Geometry: final body of the model. Coordinates: model frame, mm. A direction names the side the tool comes from. Give positions to 0.01 mm unless a question says otherwise; leave off trailing zeros. Write each loop counter-clockwise with the first axis right and the second up, starting at its lowest first coordinate (ties: lowest second). Pieces come first, ordered by that corner, then holes. Notation, with made-up numbers: (-34, 80) - (-20, 80) arc R7 ccw to (-20, 92) - close; hole circle Ø8 at (-14, 65). An arc over 180 degrees is marked (long way). One line per question, with ' | ' between items. Start each with the question number.
```python
from build123d import *

# Parameters (mm, degrees)
CHAMFER1_SIZE       = 5
SKETCH3_W           = 40
SKETCH3_H           = 200
BOSS_EXTRUDE1_DEPTH = 5
SKETCH4_W           = 500
SKETCH4_H           = 129
BOSS_EXTRUDE2_DEPTH = 10
CIRPATTERN2_COUNT   = 4


with BuildPart() as part:
    # Sketch2 → Revolve1 (revolve)
    with BuildSketch(Plane(origin=(0, 0, 0), x_dir=(1, 0, 0), z_dir=(0, 1, 0))):
        Polygon((-55.931623932, 0), (-55.931623932, 8), (-20.931623932, 8), (-20.931623932, 11), (-13.931623932, 11), (-13.931623932, 12.5), (26.068376068, 12.5), (26.068376068, 30), (568.068376068, 30), (568.068376068, 12.5), (594.068376068, 12.5), (594.068376068, 0), align=None)
    revolve(axis=Axis((0, 0, 0), (-1, 0, 0)))

    # Chamfer1
    chamfer1_edges = [part.edges().sort_by_distance(p)[0] for p in [
        (26.068376068, 0, 30),
        (568.068376068, 0, 30),
    ]]
    chamfer(chamfer1_edges, length=CHAMFER1_SIZE)

    # Sketch3 → Boss-Extrude1 (add, symmetric)
    with BuildSketch(Plane.XY):
        with Locations((139.068376068, 100)):
            Rectangle(SKETCH3_W, SKETCH3_H)
        with Locations((459.068376068, 100)):
            Rectangle(SKETCH3_W, SKETCH3_H)
    boss_extrude1 = extrude(amount=BOSS_EXTRUDE1_DEPTH, both=True)

    # Sketch4 → Boss-Extrude2 (add)
    with BuildSketch(Plane.XY.offset(5)):
        with Locations((299.068376068, 185.080398915)):
            Rectangle(SKETCH4_W, SKETCH4_H)
    boss_extrude2 = extrude(amount=BOSS_EXTRUDE2_DEPTH)

    # CirPattern2: Boss-Extrude1, Boss-Extrude2 ×4 about axis
    cirpattern2_axis = Axis((0, 0, 0), (1, 0, 0))
    add([boss_extrude1.rotate(cirpattern2_axis, i * 360 / CIRPATTERN2_COUNT) for i in range(1, CIRPATTERN2_COUNT)])
    add([boss_extrude2.rotate(cirpattern2_axis, i * 360 / CIRPATTERN2_COUNT) for i in range(1, CIRPATTERN2_COUNT)])


solid = part.part
```
1) Section D-D, the plane y = 157.5. Output: boundary loops of the cut face in (x, z), plus the area to 3 significant figures.
2) Line query: L1, parallel to Y at x = 352.5, z = -11; L2, parallel to Z at x = 252, y = 191; L3, parallel to X at y = 9.5, z = -138.5. Output: solid intervals per line, ascending.
3) Reachability of faces 5 (the flat face through (139, -76, -5)), 6 (the flat face through (296, -15, 186)), 7 (the flat face through (459, 76, 5)), 8 (the flat face through (-13.932, 10, 5)) from +Z, -Z, +X, -X, +Y, -Y: full face, straight path, thin tool, end or side. Return the list, or none.
4) Section A-A, the plane z = -48. Output: boundary loops of the cut face in (x, y).
5) First-contact query: pin 1 Ø3 at (y, z) = (-81.5, 1) entering from +X; pin 2 Ø12 at (x, z) = (458.5, 126) entering from +Y; pin 3 Ø8 at (y, z) = (166.5, 12) entering from +X; pin 4 Ø11 at (x, z) = (135.5, -1) entering from -Y. Flat tips, straight axial feed; report the tip coordinate or a pass-through.
6) Section B-B, the plane x = 507. Output: boundary loops of the cut face in (y, z).
7) Pull-direction query (Z, two-part tool) for faces 1 (the conical face through (567.826, -25.028, 3.286)), 2 (the flat face through (139, -5, 76)), 3 (the flat face through (139, 5, -76)), 4 (the flat face through (459, -116, 5)); classes: +Z half, -Z half, draft (parallel to the pull), parting line (faces both ways), or undercut.
Answer key:
1) outline: (49.07, 5) - (119.07, 5) - (119.07, -5) - (159.07, -5) - (159.07, 5) - (439.07, 5) - (439.07, -5) - (479.07, -5) - (479.07, 5) - (549.07, 5) - (549.07, 15) - (49.07, 15) - close | area: 5,800 mm^2
2) L1: -249.58 to -120.58, -27.91 to 27.91 | L2: 5 to 15 | L3: 49.07 to 549.07
3) face 5: -Z, +X, -X | face 6: +Z, +X, -X, -Y | face 7: +Z, +X, -X | face 8: -X
4) outline: (119.07, -5) - (159.07, -5) - (159.07, 5) - (119.07, 5) - close; (439.07, -5) - (479.07, -5) - (479.07, 5) - (439.07, 5) - close
5) pin 1: x = 479.07 | pin 2: y = 5 | pin 3: x = 549.07 | pin 4: y = -249.58
6) outline: (-249.58, -15) - (-120.58, -15) - (-120.58, -5) - (-249.58, -5) - close; circle Ø60 at (0, 0); (-15, 120.58) - (-5, 120.58) - (-5, 249.58) - (-15, 249.58) - close; (5, -249.58) - (15, -249.58) - (15, -120.58) - (5, -120.58) - close; (120.58, 5) - (249.58, 5) - (249.58, 15) - (120.58, 15) - close
7) face 1: parting line | face 2: undercut | face 3: undercut | face 4: +Z half
